Verification items for the finished model (mm, model axes). A direction names the side the tool comes from. Round coordinates to 2 decimals unless told otherwise and drop trailing zeros. Write each loop counter-clockwise with the first axis right and the second up, starting at its lowest first coordinate (ties: lowest second). Pieces come first, ordered by that corner, then holes.
from build123d import *

# Parameters (mm, degrees)
SKETCH1_W                                            = 60
SKETCH1_H                                            = 90
BOSS_EXTRUDE1_DEPTH                                  = 7
SKETCH2_W                                            = 60
SKETCH2_H                                            = 14
CUT_EXTRUDE1_DEPTH                                   = 2
HOLE_SIZE_PER_SOCKET_HEAD_CAP_SCREW_TYPE_D           = 6.6
HOLE_SIZE_PER_SOCKET_HEAD_CAP_SCREW_TYPE_CBORE_D     = 11
HOLE_SIZE_PER_SOCKET_HEAD_CAP_SCREW_TYPE_CBORE_DEPTH = 6.8
CHAMFER1_SIZE                                        = 1
M5_TAPPED_HOLE1_D                                    = 4.2


with BuildPart() as part:
    # Sketch1 → Boss-Extrude1 (new, symmetric)
    with BuildSketch(Plane.XY):
        Rectangle(SKETCH1_W, SKETCH1_H)
    extrude(amount=BOSS_EXTRUDE1_DEPTH, both=True)

    # Sketch2 → Cut-Extrude1 (cut)
    with BuildSketch(Plane(origin=(0, 0, -7), x_dir=(-1, 0, 0), z_dir=(0, 0, -1))):
        with Locations((0, 38)):
            Rectangle(SKETCH2_W, SKETCH2_H)
    extrude(amount=-CUT_EXTRUDE1_DEPTH, mode=Mode.SUBTRACT)

    # Hole Size per Socket Head Cap Screw Type1 (through all)
    with Locations(Plane.XY.offset(7)):
        with Locations((0, 16), (-22, 38), (22, 38), (-22, -12), (22, -38), (-22, -38), (22, -12)):
            CounterBoreHole(HOLE_SIZE_PER_SOCKET_HEAD_CAP_SCREW_TYPE_D / 2, HOLE_SIZE_PER_SOCKET_HEAD_CAP_SCREW_TYPE_CBORE_D / 2, HOLE_SIZE_PER_SOCKET_HEAD_CAP_SCREW_TYPE_CBORE_DEPTH)

    # Chamfer1
    chamfer1_edges = [part.edges().sort_by_distance(p)[0] for p in [
        (30, -45, 0),
        (-30, -45, 0),
        (-30, 45, 1),
        (30, 45, 1),
    ]]
    chamfer(chamfer1_edges, length=CHAMFER1_SIZE)

    # M5 Tapped Hole1 (through all)
    with Locations(Plane.XY.offset(7)):
        with Locations((22, 16), (-22, 16)):
            Hole(M5_TAPPED_HOLE1_D / 2)


solid = part.part
Q1. Tool access check on faces 1 (the cylindrical face through (20.81, -17.37, 3.65)), 2 (the cylindrical face through (-23.13, 17.77, -0.1)), 3 (the flat face through (0, 38, -5)). Record the directions out of +Z, -Z, +X, -X, +Y, -Y that give a thin tool (end or side, any length) a straight path to the whole face; none if there is none.
Recorded:
face 1: +Z
face 2: +Z, -Z
face 3: -Z, +X, -X, +Y
Q2. Release check for a two-part mould opening along Y. For faces 4 (the flat face through (-30, -1, 0)), 5 (the flat face through (0, 45, 1)), 6 (the cylindrical face through (2.43, 18.23, -3.45)) record: released by +Y, released by -Y, zero draft, split by the parting line, or undercut.
Recorded:
face 4: zero draft
face 5: released by +Y
face 6: undercut
Q3. Sectioned sample at C-C (x = 0). Enter the section's corners in (y, z).
Recorded:
outline: (-45, -7) - (12.7, -7) - (12.7, 0.2) - (10.5, 0.2) - (10.5, 7) - (-45, 7) - close; (19.3, -7) - (31, -7) - (31, -5) - (45, -5) - (45, 7) - (21.5, 7) - (21.5, 0.2) - (19.3, 0.2) - close
Q4. Sectioned sample at D-D (z = 5.5). Give the number of separate pieces and of enclosed holes in the cut face, plus the area to 3 significant figures.
Recorded:
separate pieces: 1
enclosed holes: 9
area: 4,710 mm2
Q5. Material ranges on line 1 along Y through (x, z) = (-22, 2); line 2 along Y through (x, z) = (-22, -1.25); line 3 along Y through (x, z) = (19, 3), recorded low to high.
Recorded:
line 1: y = -45 to -43.5, -32.5 to -17.5, -6.5 to 13.9, 18.1 to 32.5, 43.5 to 45
line 2: y = -45 to -41.3, -34.7 to -15.3, -8.7 to 13.9, 18.1 to 34.7, 41.3 to 45
line 3: y = -45 to -42.61, -33.39 to -16.61, -7.39 to 33.39, 42.61 to 45
Q6. Sectioned sample at B-B (y = 16). Enter the section's corners in (x, z).
Recorded:
outline: (-30, -7) - (-24.1, -7) - (-24.1, 7) - (-30, 7) - close; (-19.9, -7) - (-3.3, -7) - (-3.3, 0.2) - (-5.5, 0.2) - (-5.5, 7) - (-19.9, 7) - close; (3.3, -7) - (19.9, -7) - (19.9, 7) - (5.5, 7) - (5.5, 0.2) - (3.3, 0.2) - close; (24.1, -7) - (30, -7) - (30, 7) - (24.1, 7) - close
Q7. Sectioned sample at A-A (y = -38). Enter the section's corners in (x, z).
Recorded:
outline: (-30, -7) - (-25.3, -7) - (-25.3, 0.2) - (-27.5, 0.2) - (-27.5, 7) - (-30, 7) - close; (-18.7, -7) - (18.7, -7) - (18.7, 0.2) - (16.5, 0.2) - (16.5, 7) - (-16.5, 7) - (-16.5, 0.2) - (-18.7, 0.2) - close; (25.3, -7) - (30, -7) - (30, 7) - (27.5, 7) - (27.5, 0.2) - (25.3, 0.2) - close
Q8. Depth check by flat-ended pin: P1, Ø0.6, axis at x = 5.5, z = -6, coming from the +Y side; P2, Ø4, axis at x = -12, y = 34, coming from the -Z side; P3, Ø3.5, axis at x = -21.5, y = -40, coming from the +Z side. Enter the tip coordinate at first touch or a pass-through.
Recorded:
P1: stops at y = 31
P2: stops at z = -5
P3: stops at z = 0.2
